```python
from build123d import *


with BuildPart() as part:
    # Sketch1 → Revolve1 (revolve)
    with BuildSketch(Plane(origin=(0, 0, 0), x_dir=(0, 0, -1), z_dir=(1, 0, 0)), mode=Mode.PRIVATE) as revolve1_sk:
        Polygon((0, 22.5), (0, 28), (32, 28), (32, 25), (35, 25), (35, 38), (45, 38), (45, 17.5), (35, 17.5), (35, 22.5), align=None)
    revolve(revolve1_sk.sketch.rotate(Axis((0, 0, 12.011308803), (0, 0, -1)), 90), axis=Axis((0, 0, 12.011308803), (0, 0, -1)))


solid = part.part
```
CAD build for the part. Positions are in the model's coordinates, mm. A direction names the side the tool comes from. Give positions to 0.01 mm unless a question says otherwise; leave off trailing zeros. Loops run counter-clockwise (first coordinate to the right, second up) from the corner with the lowest first, then second, coordinate; pieces in that order, holes last. Notation, with made-up numbers: (65.5, 64.5) - (74.5, 64.5) arc R22 ccw to (74.5, 76.5) - close; hole circle Ø3 at (10, -24). An arc over 180 degrees is marked (long way). Put each result on its own line as item: value.
Q1. Probe line 1 along Y through (x, z) = (0, -39.75); line 2 along Z through (x, y) = (24.5, -7); line 3 along Y through (x, z) = (0, -10). List the from-to ranges inside material, lowest first.
Filled in:
line 1: y = -38 to -17.5, 17.5 to 38
line 2: z = -45 to -35, -32 to 0
line 3: y = -28 to -22.5, 22.5 to 28
Q2. Slice it at D-D (z = -37). Give the cut face in (x, y), plus the area to 3 significant figures.
Filled in:
outline: circle Ø76 at (0, 0); hole circle Ø35 at (0, 0)
area: 3,570 mm²
Q3. Slice it at C-C (z = -6.5). Give the cut face in (x, y).
Filled in:
outline: circle Ø56 at (0, 0); hole circle Ø45 at (0, 0)
Q4. Mould opens along Y. For faces 1 (the face through (-12, 13, -35)), 2 (the face through (-8.238, 37.096, -40.07)), 3 (the face through (-25, 8, -35)) say: pulls with the +Y half, pulls with the -Y half, needs draft (parallel to the pull), parting line crosses it, or undercut.
Filled in:
face 1: undercut
face 2: parting line crosses it
face 3: needs draft
Q5. Slice it at A-A (x = 0). Give the cut face in (y, z).
Filled in:
outline: (-38, -45) - (-17.5, -45) - (-17.5, -35) - (-22.5, -35) - (-22.5, 0) - (-28, 0) - (-28, -32) - (-25, -32) - (-25, -35) - (-38, -35) - close; (17.5, -45) - (38, -45) - (38, -35) - (25, -35) - (25, -32) - (28, -32) - (28, 0) - (22.5, 0) - (22.5, -35) - (17.5, -35) - close
Q6. Tool access for faces 4 (the face through (8, 16, -45)), 5 (the face through (10.382, 19.961, -17.255)), 6 (the face through (-11, -23, -32)): list every direction of +Z, -Z, +X, -X, +Y, -Y with a clear straight run to the whole face (end or side of a thin tool).
Filled in:
face 4: -Z, +X, -X, +Y, -Y
face 5: +Z
face 6: none
Q7. Flat gauge pins, fed straight in: pin 1 (6 mm diameter, centred on y = -9.5, z = -22.5, fed in from -X); pin 2 (1.5 mm diameter, centred on x = -11.5, z = -4.5, fed in from +Y); pin 3 (8 mm diameter, centred on y = -4, z = -16.5, fed in from +X); pin 4 (13.5 mm diameter, centred on x = 0.5, y = 4.5, fed in from +Z). Where does each tip first touch, or does it go through?
Filled in:
pin 1: stops at x = -27.24
pin 2: stops at y = 25.85
pin 3: stops at x = 28
pin 4: passes through
